from build123d import *

# Parameters (mm, degrees)
BASE_BODY_DEPTH            = 38
UPRIGHT_LUG_DEPTH          = 12
CENTRE_SLOT_CUT_DEPTH      = 90.397986555
CENTRE_SLOT_CUT_DEPTH_BACK = 40
SIDE_WALL_SKETCH_W         = 7
SIDE_WALL_SKETCH_H         = 22
SIDE_WALL_DEPTH            = 38
TOP_FLANGE_DEPTH           = 7
SLOT_STEP_PAD_A_SKETCH_W   = 33
SLOT_STEP_PAD_A_SKETCH_H   = 12
SLOT_STEP_PAD_A_DEPTH      = 2
SLOT_STEP_PAD_B_SKETCH_W   = 33
SLOT_STEP_PAD_B_SKETCH_H   = 12
SLOT_STEP_PAD_B_DEPTH      = 2
FLANGE_HOLES_SKETCH_R      = 4
FLANGE_HOLES_2X_8_DEPTH    = 7
LUG_BORE_SKETCH_R          = 8
LUG_BORE_16_DEPTH          = 12
LUG_HOLE_SKETCH_R          = 4
LUG_HOLE_8_DEPTH           = 12
SLOT_STEP_BLOCK_A_SKETCH_W = 33
SLOT_STEP_BLOCK_A_SKETCH_H = 12
SLOT_STEP_BLOCK_A_DEPTH    = 5
SLOT_STEP_BLOCK_B_SKETCH_W = 33
SLOT_STEP_BLOCK_B_SKETCH_H = 12
SLOT_STEP_BLOCK_B_DEPTH    = 5


with BuildPart() as part:
    # Base Profile Sketch → Base Body (new body)
    with BuildSketch(Plane.XY):
        Polygon((0, 0), (52, 0), (52, 18), (40, 18), (40, 8), (12, 8), (7, 8), (7, 18), (0, 18), align=None)
    extrude(amount=BASE_BODY_DEPTH)

    # Upright Lug Sketch → Upright Lug (add)
    with BuildSketch(Plane(origin=(52, 0, 0), x_dir=(0, 0, -1), z_dir=(1, 0, 0))):
        with BuildLine():
            Line((-38, 18), (0, 18))
            Line((0, 18), (-7.527409318, 53.518474532))
            ThreePointArc((-7.527409318, 53.518474532), (-19, 62), (-30.472590682, 53.518474532))
            Line((-30.472590682, 53.518474532), (-38, 18))
        make_face()
    extrude(amount=-UPRIGHT_LUG_DEPTH)

    # Centre Slot Sketch → Centre Slot Cut (cut, two sides: drawn at the far end of the back side and taken through both)
    with BuildSketch(Plane.ZY.offset(-CENTRE_SLOT_CUT_DEPTH_BACK)):
        Polygon((26, -144.461890512), (26, 0), (26, 12), (12, 12), (12, 0), (12, -144.461890512), (12, -433.385671535), (26, -433.385671535), align=None)
    extrude(amount=CENTRE_SLOT_CUT_DEPTH + CENTRE_SLOT_CUT_DEPTH_BACK, mode=Mode.SUBTRACT)

    # Side Wall Sketch → Side Wall (add)
    with BuildSketch(Plane.XY.offset(38)):
        with Locations((3.5, 29)):
            Rectangle(SIDE_WALL_SKETCH_W, SIDE_WALL_SKETCH_H)
    extrude(amount=-SIDE_WALL_DEPTH)

    # Top Flange Sketch → Top Flange (add)
    with BuildSketch(Plane(origin=(0, 40, 0), x_dir=(1, 0, 0), z_dir=(0, 1, 0))):
        with BuildLine():
            Line((0, 0), (-18, 0))
            ThreePointArc((-18, 0), (-20.828427125, -1.171572875), (-22, -4))
            Line((-22, -4), (-22, -34))
            ThreePointArc((-22, -34), (-20.828427125, -36.828427125), (-18, -38))
            Line((-18, -38), (0, -38))
            Line((0, -38), (0, 0))
        make_face()
    extrude(amount=-TOP_FLANGE_DEPTH)

    # Slot Step Pad A Sketch → Slot Step Pad A (add)
    with BuildSketch(Plane(origin=(0, 8, 0), x_dir=(1, 0, 0), z_dir=(0, 1, 0))):
        with Locations((23.5, -32)):
            Rectangle(SLOT_STEP_PAD_A_SKETCH_W, SLOT_STEP_PAD_A_SKETCH_H)
    extrude(amount=SLOT_STEP_PAD_A_DEPTH)

    # Slot Step Pad B Sketch → Slot Step Pad B (add)
    with BuildSketch(Plane(origin=(0, 8, 0), x_dir=(1, 0, 0), z_dir=(0, 1, 0))):
        with Locations((23.5, -6)):
            Rectangle(SLOT_STEP_PAD_B_SKETCH_W, SLOT_STEP_PAD_B_SKETCH_H)
    extrude(amount=SLOT_STEP_PAD_B_DEPTH)

    # Flange Holes Sketch → Flange Holes 2xØ8 (cut)
    with BuildSketch(Plane(origin=(0, 40, 0), x_dir=(1, 0, 0), z_dir=(0, 1, 0))):
        with Locations(Location((-9.5, -8.266515029, 0), (0, 0, 270))):
            Circle(FLANGE_HOLES_SKETCH_R)
        with Locations(Location((-9.5, -28.266515029, 0), (0, 0, 270))):
            Circle(FLANGE_HOLES_SKETCH_R)
    extrude(amount=-FLANGE_HOLES_2X_8_DEPTH, mode=Mode.SUBTRACT)

    # Lug Bore Sketch → Lug Bore Ø16 (cut)
    with BuildSketch(Plane(origin=(52, 0, 0), x_dir=(0, 0, -1), z_dir=(1, 0, 0))):
        with Locations((-19, 50)):
            Circle(LUG_BORE_SKETCH_R)
    extrude(amount=-LUG_BORE_16_DEPTH, mode=Mode.SUBTRACT)

    # Lug Hole Sketch → Lug Hole Ø8 (cut)
    with BuildSketch(Plane(origin=(52, 0, 0), x_dir=(0, 0, -1), z_dir=(1, 0, 0))):
        with Locations((-19, 30)):
            Circle(LUG_HOLE_SKETCH_R)
    extrude(amount=-LUG_HOLE_8_DEPTH, mode=Mode.SUBTRACT)

    # Slot Step Block A Sketch → Slot Step Block A (add)
    with BuildSketch(Plane(origin=(0, 10, 0), x_dir=(1, 0, 0), z_dir=(0, 1, 0))):
        with Locations((23.5, -32)):
            Rectangle(SLOT_STEP_BLOCK_A_SKETCH_W, SLOT_STEP_BLOCK_A_SKETCH_H)
    extrude(amount=SLOT_STEP_BLOCK_A_DEPTH)

    # Slot Step Block B Sketch → Slot Step Block B (add)
    with BuildSketch(Plane(origin=(0, 10, 0), x_dir=(1, 0, 0), z_dir=(0, 1, 0))):
        with Locations((23.5, -6)):
            Rectangle(SLOT_STEP_BLOCK_B_SKETCH_W, SLOT_STEP_BLOCK_B_SKETCH_H)
    extrude(amount=SLOT_STEP_BLOCK_B_DEPTH)


solid = part.part
For this review, take the finished solid that the model builds, in its own axes (mm). A direction names the side the tool comes from. Round coordinates to 2 decimals unless told otherwise and drop trailing zeros. Order: outer loops, then holes, each group sorted by start corner. A loop starts at its lowest first (then second) coordinate and runs counter-clockwise, first axis right, second up. Notation, with made-up numbers: M 60.5,86 L 67.5,86 A22 ccw 67.5,94 Z; hole C 71.25,47 d1. An arc over 180 degrees is marked long. Use a Markdown table: item, result. Add a question column.
Item 1: Add section D-D, the plane z = 29.5. Give the boundary of the cut face in (x, y).
Item 2: Add section C-C, the plane x = -9.5. Give the boundary of the cut face in (y, z), then the cut area to 3 significant figures.
Item 3: To check wall thickness, follow line 1 along X through (y, z) = (25, 4); line 2 along X through (y, z) = (39.5, 30); line 3 along Y through (x, z) = (45, 19). State the ranges of each line that lie inside material, in increasing order.
Item 4: Add section A-A, the plane x = 35. Give the boundary of the cut face in (y, z).
Item 5: Add section B-B, the plane y = 16.5. Give the boundary of the cut face in (x, z).
Item 6: Mouldability with a two-part tool opening along Z and no side actions: class faces 1 (the flat face through (46.08, 35.51, 3.71)), 2 (the flat face through (40, 25, 19)), 3 (the flat face through (23, 15, 32)), 4 (the flat face through (46.084, 36.008, 34.184)) as released by +Z, released by -Z, zero draft, split by the parting line, or undercut.
Item 7: Insertion check: pin 1 (9 mm diameter, centred on x = -9.5, z = 8.27, fed in from +Y); pin 2 (16.5 mm diameter, centred on y = 23.5, z = 27.5, fed in from -X); pin 3 (1.5 mm diameter, centred on x = 1, z = 20, fed in from -Y); pin 4 (10 mm diameter, centred on x = 34.5, y = 45, fed in from -Z). Each pin has a flat end and moves straight along its axis. Give the tip position at first contact, or say it passes through.
Item 8: Tool access review of faces 5 (the flat face through (23, 15, 6)), 6 (the cylindrical face through (46.084, 33.966, 19.521)), 7 (the flat face through (20, 7, 26)), 8 (the flat face through (-8, 40, 19)): name each direction out of +Z, -Z, +X, -X, +Y, -Y from which nothing blocks a thin tool from reaching the whole face with its end or side.
Geometry results:
| question | item | result |
|---|---|---|
| 1 | outline | M -22,33 L -13.31,33 L -13.31,40 L -22,40 Z; M -5.69,33 L 0,33 L 0,0 L 52,0 L 52,55.81 L 40,55.81 L 40,15 L 7,15 L 7,40 L -5.69,40 Z |
| 2 | outline | M 33,0 L 40,0 L 40,4.27 L 33,4.27 Z; M 33,12.27 L 40,12.27 L 40,24.27 L 33,24.27 Z; M 33,32.27 L 40,32.27 L 40,38 L 33,38 Z |
| 2 | area | 154 mm² |
| 3 | line 1 | x = 0 to 7, 40 to 52 |
| 3 | line 2 | x = -22 to -13.1, -5.9 to 7, 40 to 52 |
| 3 | line 3 | y = 0 to 26, 34 to 42, 58 to 62 |
| 4 | outline | M 0,0 L 15,0 L 15,12 L 0,12 Z; M 0,26 L 15,26 L 15,38 L 0,38 Z |
| 5 | outline | M 0,0 L 7,0 L 7,38 L 0,38 Z; M 40,0 L 52,0 L 52,38 L 40,38 Z |
| 6 | face 1 | released by -Z |
| 6 | face 2 | undercut |
| 6 | face 3 | zero draft |
| 6 | face 4 | released by +Z |
| 7 | pin 1 | stops at y = 40 |
| 7 | pin 2 | stops at x = 0 |
| 7 | pin 3 | stops at y = 12 |
| 7 | pin 4 | passes through |
| 8 | face 5 | +Z, -Z, +Y |
| 8 | face 6 | +X |
| 8 | face 7 | -Y |
| 8 | face 8 | +Z, -Z, -X, +Y |
